from build123d import *

# Parameters (mm, degrees)
BOSS_EXTRUDE1_DEPTH = 6
SKETCH2_R           = 3.5
CUT_EXTRUDE1_DEPTH  = 95


with BuildPart() as part:
    # Sketch1 → Boss-Extrude1 (new body)
    with BuildSketch(Plane.XY):
        with BuildLine():
            Line((0, 10), (57.02, 10))
            ThreePointArc((57.02, 10), (67.02, 0), (57.02, -10))
            Line((57.02, -10), (0, -10))
            ThreePointArc((0, -10), (-10, 0), (0, 10))
        make_face()
    extrude(amount=BOSS_EXTRUDE1_DEPTH)

    # Sketch2 → Cut-Extrude1 (cut)
    with BuildSketch(Plane.XY.offset(6)):
        Circle(SKETCH2_R)
        with Locations((57.02, 0)):
            Circle(SKETCH2_R)
    extrude(amount=-CUT_EXTRUDE1_DEPTH, mode=Mode.SUBTRACT)


solid = part.part
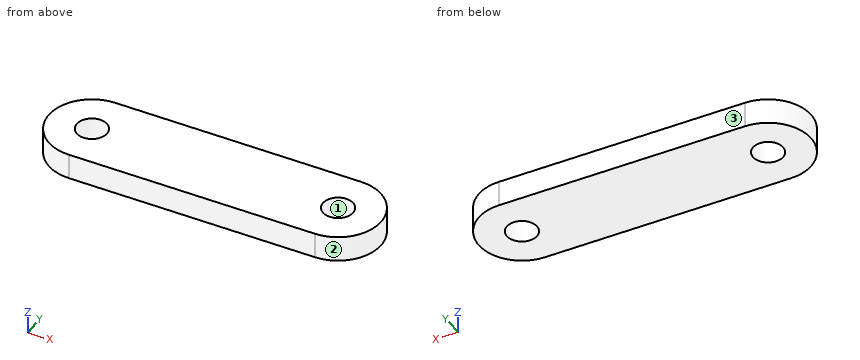
The model under review builds one solid part; all positions refer to its coordinate system, in mm. Face numbers are marked on the shaded views. Round coordinates to 2 decimals unless told otherwise and drop trailing zeros. Loops run counter-clockwise (first coordinate to the right, second up) from the corner with the lowest first, then second, coordinate; pieces in that order, holes last. Notation, with made-up numbers: (70.25, 6.5) -> (127.25, 6.5) arc R17 cw to (127.25, 38.5) -> close; hole circle Ø4 at (9.5, 66.25). An arc over 180 degrees is marked (long way). Return JSON: item names as keys, results as strings.
(1) Add section A-A on z = 5.3. Write out the cut boundary in (x, y), plus the area to 3 significant figures.
Solved:
{"outline": "(0, -10) -> (57.02, -10) arc R10 ccw to (57.02, 10) -> (0, 10) arc R10 ccw to start; hole circle Ø7 at (0, 0); hole circle Ø7 at (57.02, 0)", "area": "1,380 mm2"}
(2) The part is to be moulded in two halves that separate along X. For the marked faces 1, 2 and 3, say which applies: released by +X, released by -X, zero draft, split by the parting line, or undercut.
Solved:
{"face 1": "undercut", "face 2": "released by +X", "face 3": "zero draft"}
(3) For line 1 (Y direction, x = 0, z = 4.2); line 2 (X direction, y = 2.25, z = 5.15); line 3 (X direction, y = -2, z = 0.9), list the stretches that pass through material, from the lowest coordinate up.
Solved:
{"line 1": "-10 to -3.5, 3.5 to 10", "line 2": "-9.74 to -2.68, 2.68 to 54.34, 59.7 to 66.76", "line 3": "-9.8 to -2.87, 2.87 to 54.15, 59.89 to 66.82"}
(4) Add section C-C on x = 54.5. Write out the cut boundary in (y, z), plus the area to 3 significant figures.
Solved:
{"outline": "(-10, 0) -> (-2.43, 0) -> (-2.43, 6) -> (-10, 6) -> close; (2.43, 0) -> (10, 0) -> (10, 6) -> (2.43, 6) -> close", "area": "90.9 mm2"}
(5) Add section B-B on y = 0. Write out the cut boundary in (x, z).
Solved:
{"outline": "(-10, 0) -> (-3.5, 0) -> (-3.5, 6) -> (-10, 6) -> close; (3.5, 0) -> (53.52, 0) -> (53.52, 6) -> (3.5, 6) -> close; (60.52, 0) -> (67.02, 0) -> (67.02, 6) -> (60.52, 6) -> close"}
(6) Add section D-D on y = -4.75. Write out the cut boundary in (x, z).
Solved:
{"outline": "(-8.8, 0) -> (65.82, 0) -> (65.82, 6) -> (-8.8, 6) -> close"}
